from build123d import *

# Parameters (mm, degrees)
SKETCH_1_R              = 12.5
EXTRUDE_1_DEPTH         = 440
CHAMFER_1_SIZE          = 1
HOLE_WIZARD_M10_1_D     = 8.5
HOLE_WIZARD_M10_1_DEPTH = 26.5
HOLE_WIZARD_M10_1_TIP   = 2.553657631


with BuildPart() as part:
    # 草图1 → 凸台-拉伸1 (new body)
    with BuildSketch(Plane(origin=(0, 0, 0), x_dir=(1, 0, 0), z_dir=(0, 1, 0))):
        with Locations(Location((0, 0, 0), (0, 0, 270))):
            Circle(SKETCH_1_R)
    extrude(amount=EXTRUDE_1_DEPTH)

    # 倒角1
    chamfer_1_edges = [part.edges().sort_by_distance(p)[0] for p in [
        (0, 0, -12.5),
        (0, 440, -12.5),
    ]]
    chamfer(chamfer_1_edges, length=CHAMFER_1_SIZE)

    # M10 螺纹孔1
    with Locations(Plane(origin=(0, 440, 0), x_dir=(1, 0, 0), z_dir=(0, 1, 0))):
        with Locations((0, 0)):
            Hole(HOLE_WIZARD_M10_1_D / 2, depth=HOLE_WIZARD_M10_1_DEPTH)
            with Locations((0, 0, -(HOLE_WIZARD_M10_1_DEPTH + HOLE_WIZARD_M10_1_TIP / 2))):  # 118° drill point
                Cone(0, HOLE_WIZARD_M10_1_D / 2, HOLE_WIZARD_M10_1_TIP, mode=Mode.SUBTRACT)


solid = part.part
The model under review builds one solid part; all positions refer to its coordinate system, in mm. Round coordinates to 2 decimals unless told otherwise and drop trailing zeros. Write each loop counter-clockwise with the first axis right and the second up, starting at its lowest first coordinate (ties: lowest second). Pieces come first, ordered by that corner, then holes. Notation, with made-up numbers: M 9,-37 L 24,-37 A6 ccw 24,-31 Z; hole C 75.25,7.5 d11. An arc over 180 degrees is marked long. Use a Markdown table: item, result. Add a question column.
Q1. To check wall thickness, follow line 1 (Z direction, x = -0.5, y = 335); line 2 (X direction, y = 204, z = 10.75); line 3 (X direction, y = 54.5, z = 4.75). State the ranges of each line that lie inside material, in increasing order.
Q2. Insertion check: pin 1 (6 mm diameter, centred on y = 310, z = -6.5, fed in from +X); pin 2 (12 mm diameter, centred on y = 247.5, z = -7.5, fed in from -X); pin 3 (4 mm diameter, centred on y = 342.5, z = 9.5, fed in from +X). Each pin has a flat end and moves straight along its axis. Give the tip position at first contact, or say it passes through.
Q3. The part is to be moulded in two halves that separate along X. For faces 1 (the face through (-2.285, 426.564, -3.584)), 2 (the face through (0, 0, 0)), 3 (the face through (3.755, 216.934, 11.923)), say which applies: pulls with the +X half, pulls with the -X half, needs draft (parallel to the pull), parting line crosses it, or undercut.
Q4. We need section A-A, the plane y = 109.5. State the section outline as (x, z) points.
Findings below:
| question | item | result |
|---|---|---|
| 1 | line 1 | z = -12.49 to 12.49 |
| 1 | line 2 | x = -6.38 to 6.38 |
| 1 | line 3 | x = -11.56 to 11.56 |
| 2 | pin 1 | stops at x = 12 |
| 2 | pin 2 | stops at x = -12.41 |
| 2 | pin 3 | stops at x = 10 |
| 3 | face 1 | undercut |
| 3 | face 2 | needs draft |
| 3 | face 3 | parting line crosses it |
| 4 | outline | C 0,0 d25 |
